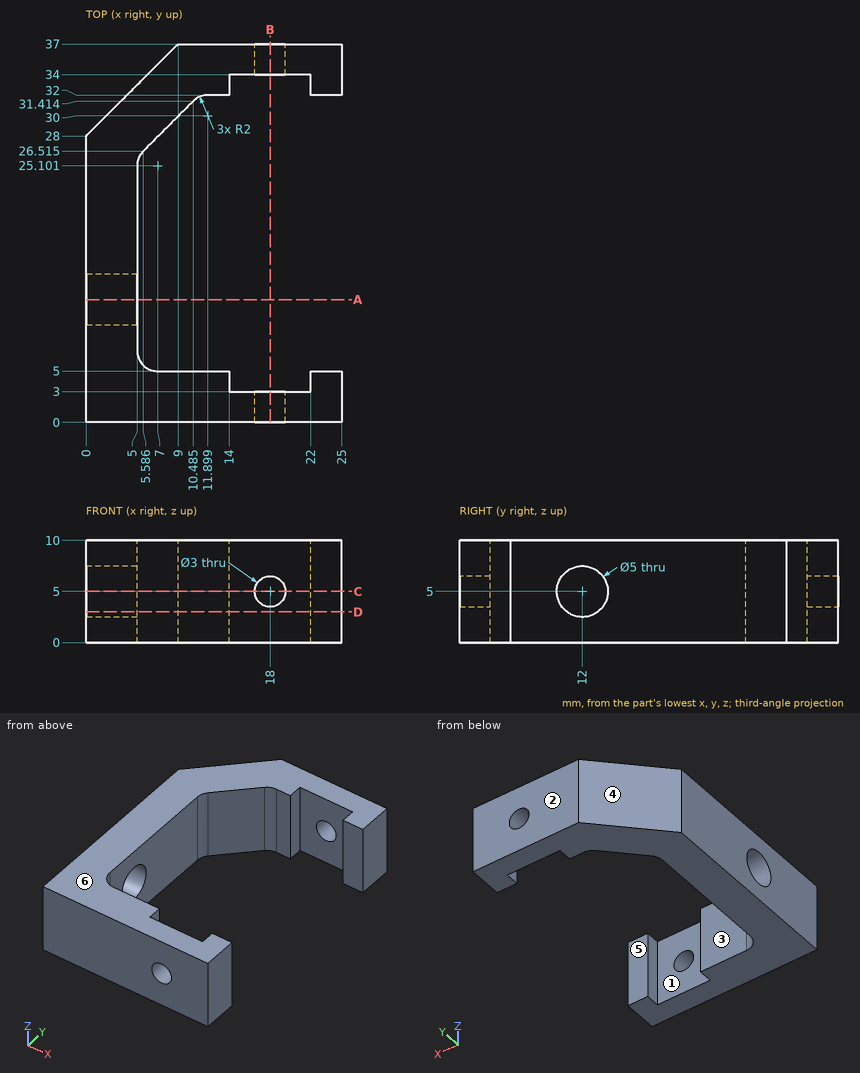
Here's the drawing with two shaded views (mm, measured from the low corner). I have some questions. A direction names the side the tool comes from. Give positions to 0.01 mm unless a question says otherwise; leave off trailing zeros. Write each loop counter-clockwise with the first axis right and the second up, starting at its lowest first coordinate (ties: lowest second). Pieces come first, ordered by that corner, then holes. Notation, with made-up numbers: (6.5, 82.25) - (41.5, 82.25) arc R19 ccw to (41.5, 113.25) - close; hole circle Ø5 at (59, 17.5). An arc over 180 degrees is marked (long way). One line per item, written item: value. Start each with the question number.
Item 1: If we mould it in two halves opening along Y, with no side actions, what happens to the marked faces 4, 5 and 6? For each: +Y half, -Y half, draft (parallel to the pull), parting line (faces both ways), or undercut.
Item 2: Please list where these lines run through material, in increasing order: line 1 (Y direction, x = 22.5, z = 4); line 2 (Y direction, x = 20.5, z = 7); line 3 (X direction, y = 35, z = 5). Write a range as from..to.
Item 3: Imagine slicing it at A-A, the plane y = 12. List the corners of the cut face in (x, z) for me, and give its area (3 significant figures).
Item 4: Which directions (+Z, -Z, +X, -X, +Y, -Y) give clear straight access to the entire face, cutting with the end or side of a thin tool? Please do the marked faces 1, 2 and 3.
Item 5: Imagine slicing it at D-D, the plane z = 3. List the corners of the cut face in (x, y) for me (1 decimal).
Item 6: I'm going to push flat-ended pins straight in: pin 1 (3 mm diameter, centred on y = 29, z = 7.5, fed in from +X); pin 2 (6 mm diameter, centred on y = 14, z = 7, fed in from -X); pin 3 (6 mm diameter, centred on y = 12, z = 5, fed in from +X); pin 4 (2 mm diameter, centred on y = 33.5, z = 2.5, fed in from -X). Where does each tip first touch, or does it pass through?
Item 7: Imagine slicing it at C-C, the plane z = 5. Give the number of separate pieces and of enclosed holes in the cut face, and give its area (3 significant figures).
Item 8: Imagine slicing it at B-B, the plane x = 18. List the corners of the cut face in (y, z) for me.
Geometry says:
1. face 4: +Y half
1. face 5: undercut
1. face 6: draft
2. line 1: 0..5, 32..37
2. line 2: 0..3, 34..37
2. line 3: 7..16.5, 19.5..25
3. outline: (0, 0) - (5, 0) - (5, 2.5) - (0, 2.5) - close; (0, 7.5) - (5, 7.5) - (5, 10) - (0, 10) - close
3. area: 25.0 mm^2
4. face 1: +Z, -Z
4. face 2: +Z, -Z, +X, -X, +Y
4. face 3: +Z, -Z, +X
5. outline: (0, 0) - (25, 0) - (25, 5) - (22, 5) - (22, 3) - (14, 3) - (14, 5) - (7, 5) arc R2 cw to (5, 7) - (5, 10.5) - (0, 10.5) - close; (0, 13.5) - (5, 13.5) - (5, 25.1) arc R2 cw to (5.6, 26.5) - (10.5, 31.4) arc R2 cw to (11.9, 32) - (14, 32) - (14, 34) - (22, 34) - (22, 32) - (25, 32) - (25, 37) - (9, 37) - (0, 28) - close
6. pin 1: x = 9.57
6. pin 2: x = 0
6. pin 3: x = 5
6. pin 4: x = 4.5
7. separate pieces: 4
7. enclosed holes: 0
7. area: 289 mm^2
8. outline: (0, 0) - (3, 0) - (3, 3.5) - (0, 3.5) - close; (0, 6.5) - (3, 6.5) - (3, 10) - (0, 10) - close; (34, 0) - (37, 0) - (37, 3.5) - (34, 3.5) - close; (34, 6.5) - (37, 6.5) - (37, 10) - (34, 10) - close
